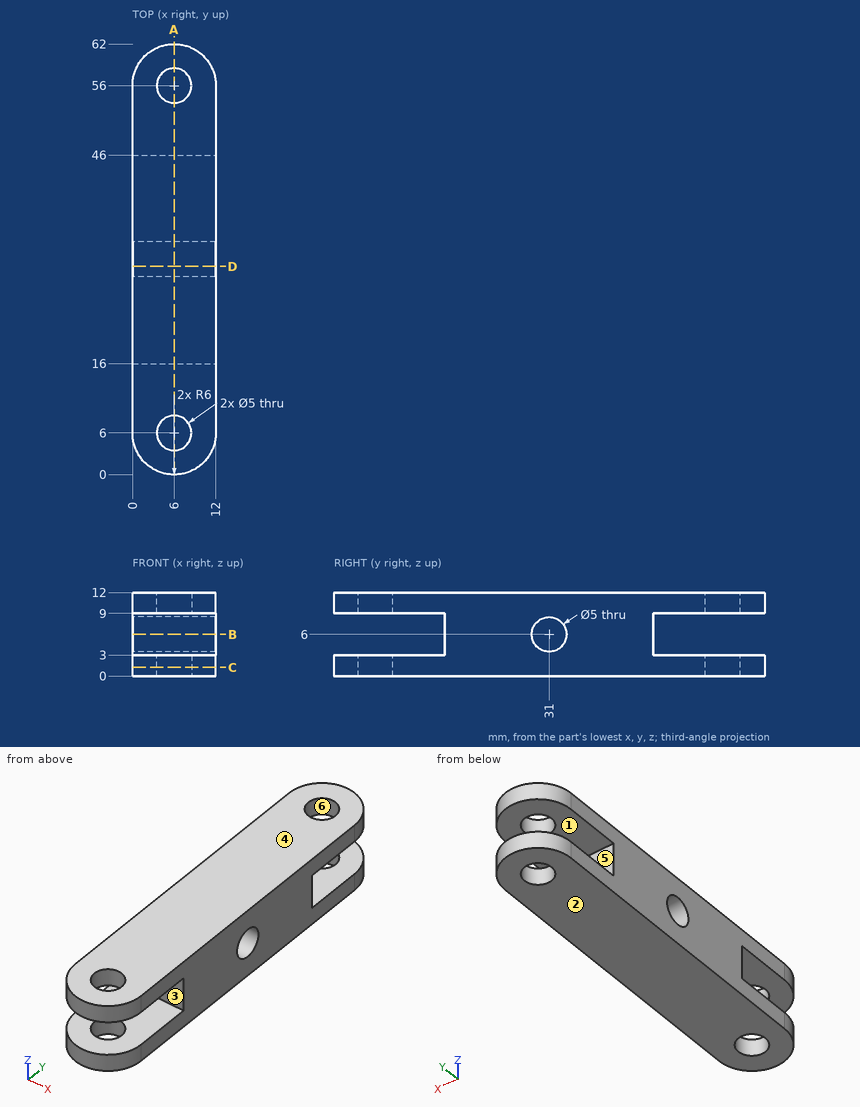
Verification items for this drawing (mm, ordinates from the low corner). A direction names the side the tool comes from. Give positions to 0.01 mm unless a question says otherwise; leave off trailing zeros. Write each loop counter-clockwise with the first axis right and the second up, starting at its lowest first coordinate (ties: lowest second). Pieces come first, ordered by that corner, then holes.
1) Access from +Z, -Z, +X, -X, +Y, -Y to the whole of each face (thin tool, end or side, straight path). Record for the marked faces 1, 2 and 3.
2) Section check B-B, the plane z = 6. Record the boundary of the cut face in (x, y).
3) Section check A-A, the plane x = 6. State how many separate pieces and enclosed holes the cut face has, and give its area (3 significant figures).
4) Release check for a two-part mould opening along Y. For the marked faces 4, 5 and 6 record: pulls with the +Y half, pulls with the -Y half, needs draft (parallel to the pull), parting line crosses it, or undercut.
5) Material ranges on L1, parallel to Y at x = 6.25, z = 10; L2, parallel to Z at x = 9.25, y = 46.5; L3, parallel to Y at x = 9.25, z = 6, recorded low to high.
6) Gauge pin test, flat ends, axial feed: pin 1 (1.8 mm diameter, centred on x = 3.5, z = 5, fed in from +Y); pin 2 (5 mm diameter, centred on x = 9, z = 2, fed in from +Y). Record the tip position at first contact, or that the pin passes through.
7) Section check C-C, the plane z = 1.25. Record the boundary of the cut face in (x, y).
8) Section check D-D, the plane y = 30. Record the boundary of the cut face in (x, z), and give its area (3 significant figures).
Computed:
1. face 1: +X, -X, +Y
1. face 2: -Z, +X, -X, +Y, -Y
1. face 3: +X, -X, -Y
2. outline: (0, 16) - (12, 16) - (12, 28.5) - (0, 28.5) - close; (0, 33.5) - (12, 33.5) - (12, 46) - (0, 46) - close
3. separate pieces: 5
3. enclosed holes: 1
3. area: 472 mm2
4. face 4: needs draft
4. face 5: pulls with the +Y half
4. face 6: undercut
5. L1: y = 0.01 to 3.51, 8.49 to 53.51, 58.49 to 61.99
5. L2: z = 0 to 3, 9 to 12
5. L3: y = 16 to 28.5, 33.5 to 46
6. pin 1: stops at y = 46
6. pin 2: stops at y = 61.98
7. outline: (0, 6) arc R6 ccw to (12, 6) - (12, 56) arc R6 ccw to (0, 56) - close; hole circle Ø5 at (6, 6); hole circle Ø5 at (6, 56)
8. outline: (0, 0) - (12, 0) - (12, 3.71) - (0, 3.71) - close; (0, 8.29) - (12, 8.29) - (12, 12) - (0, 12) - close
8. area: 89.0 mm2
